Geometry: see drawing. Coordinates: mm, zero at the bounding-box minimum. Give positions to 0.01 mm unless a question says otherwise; leave off trailing zeros. Write each loop counter-clockwise with the first axis right and the second up, starting at its lowest first coordinate (ties: lowest second). Pieces come first, ordered by that corner, then holes. Notation, with made-up numbers: (27.5, 27.25) -> (67.5, 27.25) arc R29 ccw to (67.5, 60.25) -> close; hole circle Ø7 at (85, -34.75). An arc over 180 degrees is marked (long way). Use one line per item in the form item = value. Start each with the question number.
(1) Cut plane C-C, the plane x = 24. Output: boundary loops of the cut face in (y, z), and give its area (3 significant figures).
(2) Cut plane A-A, the plane y = 17.75. Output: boundary loops of the cut face in (x, z), and give its area (3 significant figures).
(3) Cut plane B-B, the plane z = 194. Output: boundary loops of the cut face in (x, y).
(4) First-contact query: P1, Ø4, axis at y = 12, z = 26.5, coming from the -X side; P2, Ø3, axis at y = 26, z = 109, coming from the -X side (1 decimal); P3, Ø8, axis at y = 18.5, z = 75.5, coming from the -X side. Flat tips, straight axial feed; report the tip coordinate or a pass-through.
(5) Material intervals for line 1 along X through (y, z) = (28, 148.5) (1 decimal); line 2 along X through (y, z) = (15.75, 146); line 3 along Z through (x, y) = (56, 4) (1 decimal), sorted ascending. Write a range as from..to.
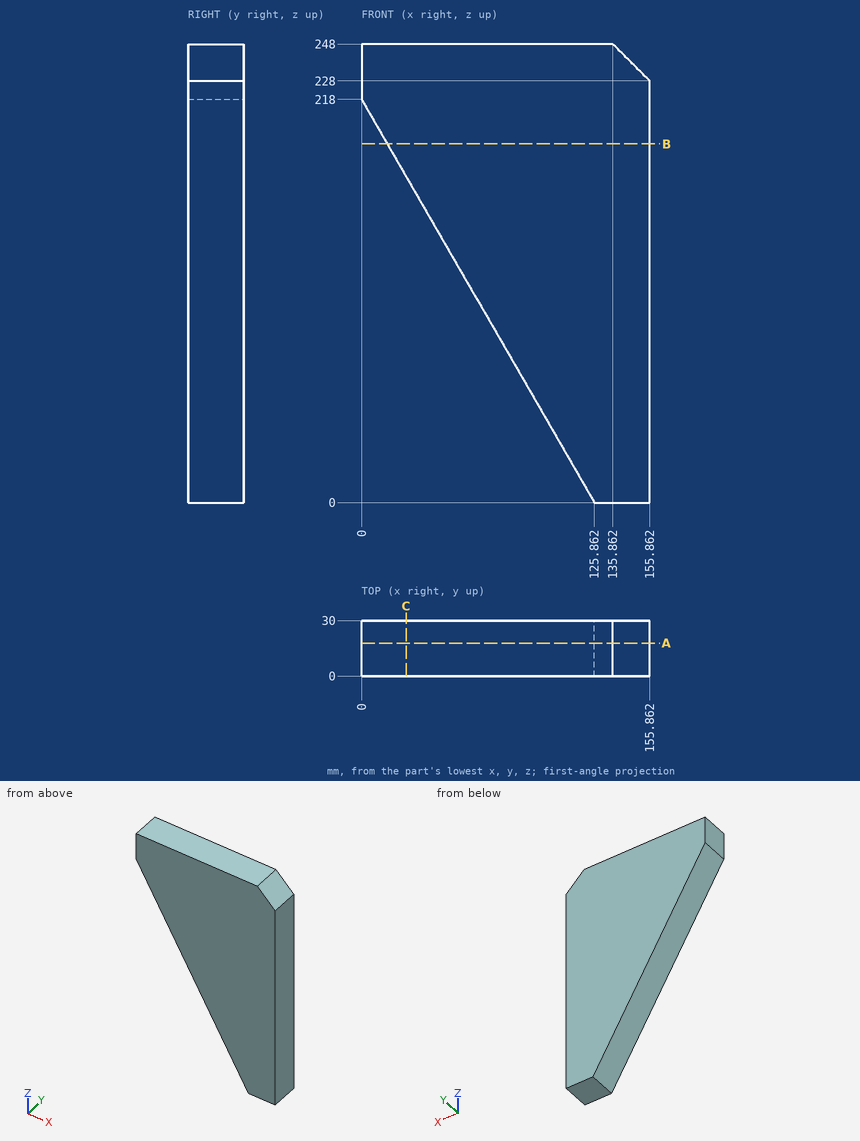
Geometry says:
q1.outline = (0, 176.43) -> (30, 176.43) -> (30, 248) -> (0, 248) -> close
q1.area = 2,150 mm^2
q2.outline = (0, 218) -> (125.86, 0) -> (155.86, 0) -> (155.86, 228) -> (135.86, 248) -> (0, 248) -> close
q2.area = 24,700 mm^2
q3.outline = (13.86, 0) -> (155.86, 0) -> (155.86, 30) -> (13.86, 30) -> close
q4.P1 = 109.41
q4.P2 = 62.1
q4.P3 = 79.96
q5.line_1 = 40.1..155.9
q5.line_2 = 41.57..155.86
q5.line_3 = 121..248
